Here's the drawing with two shaded views (mm, measured from the low corner). I have some questions. A direction names the side the tool comes from. Coordinates: 2 decimals unless noted, no trailing zeros. Order: outer loops, then holes, each group sorted by start corner. A loop starts at its lowest first (then second) coordinate and runs counter-clockwise, first axis right, second up. Notation, with made-up numbers: (54, 22) - (78, 22) arc R34 ccw to (78, 52) - close; hole circle Ø9 at (7.5, 71). An arc over 180 degrees is marked (long way). One line per item, written item: value. Start each with the question number.
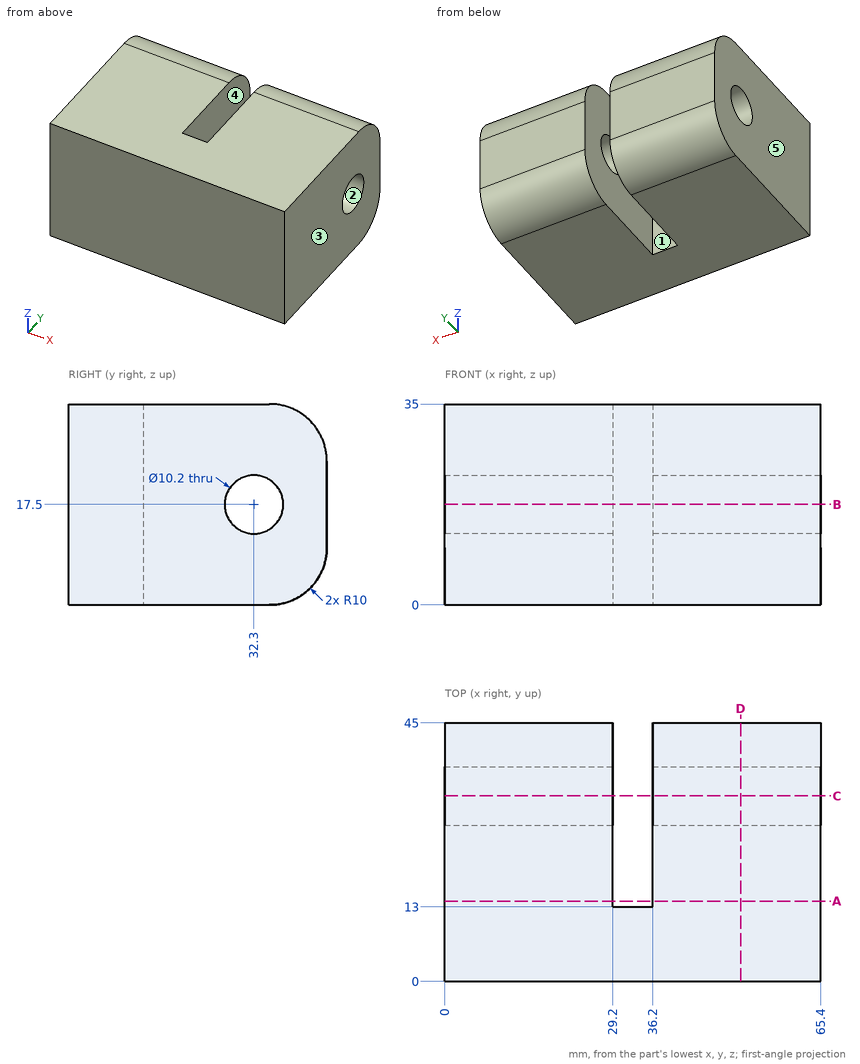
Q1. I want a section at A-A on y = 14. Please give me the cut outline in (x, z).
Q2. If I drill on L1, parallel to X at y = 21, z = 22; L2, parallel to Y at x = 51, z = 17.5; L3, parallel to Z at x = 48.5, y = 36, over which ranges is the centre line in solid material (lowest first)?
Q3. I'm going to push flat-ended pins straight in: pin 1 (16 mm diameter, centred on y = 29, z = 9.5, fed in from -X); pin 2 (9 mm diameter, centred on y = 32.3, z = 17.5, fed in from +X). Where does each tip first touch, or does it pass through?
Q4. I want a section at C-C on y = 32.3. Please give me the cut outline in (x, z).
Q5. I want a section at B-B on z = 17.5. Please give me the cut outline in (x, y).
Q6. We'd pull the mould along X, two halves only. Please class the marked faces 3, 4 and 5: +X half, -X half, draft (parallel to the pull), parting line (faces both ways), or undercut.
Q7. I want a section at D-D on x = 51.5. Please give me the cut outline in (y, z), then the cut area to 3 significant figures.
Q8. Which directions (+Z, -Z, +X, -X, +Y, -Y) give clear straight access to the entire face, cutting with the end or side of a thin tool? Please do the marked faces 1 and 2.
Values follow:
1. outline: (0, 0) - (29.2, 0) - (29.2, 35) - (0, 35) - close; (36.2, 0) - (65.4, 0) - (65.4, 35) - (36.2, 35) - close
2. L1: x = 0 to 29.2, 36.2 to 65.4
2. L2: y = 0 to 27.2, 37.4 to 45
2. L3: z = 0.05 to 13.99, 21.01 to 34.95
3. pin 1: stops at x = 0
3. pin 2: passes through
4. outline: (0, 0) - (29.2, 0) - (29.2, 12.4) - (0, 12.4) - close; (0, 22.6) - (29.2, 22.6) - (29.2, 35) - (0, 35) - close; (36.2, 0) - (65.4, 0) - (65.4, 12.4) - (36.2, 12.4) - close; (36.2, 22.6) - (65.4, 22.6) - (65.4, 35) - (36.2, 35) - close
5. outline: (0, 0) - (65.4, 0) - (65.4, 27.2) - (36.2, 27.2) - (36.2, 13) - (29.2, 13) - (29.2, 27.2) - (0, 27.2) - close; (0, 37.4) - (29.2, 37.4) - (29.2, 45) - (0, 45) - close; (36.2, 37.4) - (65.4, 37.4) - (65.4, 45) - (36.2, 45) - close
6. face 3: +X half
6. face 4: undercut
6. face 5: -X half
7. outline: (0, 0) - (35, 0) arc R10 ccw to (45, 10) - (45, 25) arc R10 ccw to (35, 35) - (0, 35) - close; hole circle Ø10.2 at (32.3, 17.5)
7. area: 1,450 mm^2
8. face 1: +Z, -Z, +Y
8. face 2: +X, -X
